```python
from build123d import *

# Parameters (mm, degrees)
SKETCH1_W                  = 80
SKETCH1_H                  = 330
BOSS_EXTRUDE1_DEPTH        = 10
F_6_6_6_6_DIAMETER_HOLE1_D = 6.6
CUT_EXTRUDE1_DEPTH         = 10


with BuildPart() as part:
    # Sketch1 → Boss-Extrude1 (new body)
    with BuildSketch(Plane(origin=(0, 0, 0), x_dir=(1, 0, 0), z_dir=(0, 1, 0))):
        Rectangle(SKETCH1_W, SKETCH1_H)
    extrude(amount=BOSS_EXTRUDE1_DEPTH)

    # Ø6.6 (6.6) Diameter Hole1 (through all)
    with Locations(Plane(origin=(0, 10, 0), x_dir=(1, 0, 0), z_dir=(0, 1, 0))):
        with Locations((-25, -80), (25, -80)):
            Hole(F_6_6_6_6_DIAMETER_HOLE1_D / 2)

    # Sketch5 → Cut-Extrude1 (cut)
    with BuildSketch(Plane(origin=(0, 10, 0), x_dir=(1, 0, 0), z_dir=(0, 1, 0))):
        with BuildLine():
            Line((-28.3, 97.5), (-28.3, 122.5))
            ThreePointArc((-28.3, 122.5), (-25, 125.8), (-21.7, 122.5))
            Line((-21.7, 122.5), (-21.7, 97.5))
            ThreePointArc((-21.7, 97.5), (-25, 94.2), (-28.3, 97.5))
        make_face()
        with BuildLine():
            Line((21.7, 97.5), (21.7, 122.5))
            ThreePointArc((21.7, 122.5), (25, 125.8), (28.3, 122.5))
            Line((28.3, 122.5), (28.3, 97.5))
            ThreePointArc((28.3, 97.5), (25, 94.2), (21.7, 97.5))
        make_face()
    extrude(amount=-CUT_EXTRUDE1_DEPTH, mode=Mode.SUBTRACT)


solid = part.part
```
Verification items for the finished model (mm, model axes). A direction names the side the tool comes from. Give positions to 0.01 mm unless a question says otherwise; leave off trailing zeros. Write each loop counter-clockwise with the first axis right and the second up, starting at its lowest first coordinate (ties: lowest second). Pieces come first, ordered by that corner, then holes. Notation, with made-up numbers: M -0.5,34 L 45.5,34 A24 cw 45.5,57 Z; hole C 74,10.25 d5. An arc over 180 degrees is marked long. One line per question, with ' | ' between items.
1) Thickness scan on line 1 along X through (y, z) = (6.5, 80); line 2 along Z through (x, y) = (25, 7); line 3 along Z through (x, y) = (27.5, 4.75). Record the ranges inside material, lowest first. Write a range as [from, to].
Result:
line 1: x = [-40, -28.3], [-21.7, 21.7], [28.3, 40] | line 2: z = [-165, -125.8], [-94.2, 76.7], [83.3, 165] | line 3: z = [-165, -124.65], [-95.35, 77.85], [82.15, 165]
2) Section check B-B on z = 80. Enter the section's corners in (x, y), plus the area to 3 significant figures.
Result:
outline: M -40,0 L -28.3,0 L -28.3,10 L -40,10 Z; M -21.7,0 L 21.7,0 L 21.7,10 L -21.7,10 Z; M 28.3,0 L 40,0 L 40,10 L 28.3,10 Z | area: 668 mm2
3) Set-up check for faces 4 (the cylindrical face through (24.9, 5.1, -125.8)), 5 (the flat face through (-1, 10, -2)): record each of +Z, -Z, +X, -X, +Y, -Y from which the full face is reachable in a straight line by a thin tool's end or side.
Result:
face 4: +Y, -Y | face 5: +Z, -Z, +X, -X, +Y
4) Mould release check, pull along Z, two halves, no side actions. Record for faces 1 (the flat face through (-1, 0, -2)), 2 (the cylindrical face through (-24.9, 5.1, -94.2)), 3 (the flat face through (-1, 5, 165)): released by +Z, released by -Z, zero draft, split by the parting line, or undercut.
Result:
face 1: zero draft | face 2: undercut | face 3: released by +Z
5) Section check C-C on y = 4. Enter the section's corners in (x, z), plus the area to 3 significant figures.
Result:
outline: M -40,-165 L 40,-165 L 40,165 L -40,165 Z; hole M -28.3,-122.5 A3.3 ccw -21.7,-122.5 L -21.7,-97.5 A3.3 ccw -28.3,-97.5 Z; hole C -25,80 d6.6; hole M 21.7,-122.5 A3.3 ccw 28.3,-122.5 L 28.3,-97.5 A3.3 ccw 21.7,-97.5 Z; hole C 25,80 d6.6 | area: 25,900 mm2
6) Section check A-A on x = -25. Enter the section's corners in (y, z), plus the area to 3 significant figures.
Result:
outline: M 0,-165 L 10,-165 L 10,-125.8 L 0,-125.8 Z; M 0,-94.2 L 10,-94.2 L 10,76.7 L 0,76.7 Z; M 0,83.3 L 10,83.3 L 10,165 L 0,165 Z | area: 2,920 mm2
7) Gauge pin test, flat ends, axial feed: pin 1 Ø10 at (x, z) = (-27, -52) entering from -Y; pin 2 Ø5.5 at (x, z) = (-25, 80) entering from +Y. Record the tip position at first contact, or that the pin passes through.
Result:
pin 1: stops at y = 0 | pin 2: passes through
